```python
from build123d import *

# Parameters (mm, degrees)
BLOCK_BODY_2IN_DEPTH                      = 50.8
SIDE_THROUGH_HOLE_0_234_D                 = 5.9436
SIDE_HOLE_EDGE_CHAMFER_SIZE               = 0.635
DOWEL_HOLE_0_126_D                        = 3.2004
DOWEL_HOLE_0_126_DEPTH                    = 6.0198
DOWEL_HOLE_0_126_TIP                      = 1.6002
COUNTERSUNK_SCREW_HOLE_NO0_D              = 6.7564
COUNTERSUNK_SCREW_HOLE_NO0_CSINK_D        = 13.208
COUNTERSUNK_SCREW_HOLE_NO0_CSINK_ANGLE    = 82
COUNTERBORED_BOLT_HOLE_0_25IN_D           = 6.7564
COUNTERBORED_BOLT_HOLE_0_25IN_CBORE_D     = 11.176
COUNTERBORED_BOLT_HOLE_0_25IN_CBORE_DEPTH = 6.35


with BuildPart() as part:
    # Block Profile Sketch → Block Body 2in (new body)
    with BuildSketch(Plane.XY):
        Polygon((0, 12.7), (19.05, 12.7), (19.05, -31.75), (0, -31.75), (0, 0), (-15.875, 0), (-15.875, 12.7), align=None)
    extrude(amount=BLOCK_BODY_2IN_DEPTH)

    # Side Through Hole Ø0.234 (through all)
    with Locations(Plane(origin=(0, -15.875, 25.4), x_dir=(0, -1, 0), z_dir=(-1, 0, 0))):
        with Locations((0, 0)):
            Hole(SIDE_THROUGH_HOLE_0_234_D / 2)

    # Side Hole Edge Chamfer
    side_hole_edge_chamfer_edges = [part.edges().sort_by_distance(p)[0] for p in [
        (0, -18.8468, 25.4),
        (19.05, -18.8468, 25.4),
    ]]
    chamfer(side_hole_edge_chamfer_edges, length=SIDE_HOLE_EDGE_CHAMFER_SIZE)

    # Dowel Hole Ø0.126
    with Locations(Plane(origin=(-7.9375, 0, 25.4), x_dir=(-1, 0, 0), z_dir=(0, -1, 0))):
        with Locations((0, 0)):
            Hole(DOWEL_HOLE_0_126_D / 2, depth=DOWEL_HOLE_0_126_DEPTH)
            with Locations((0, 0, -(DOWEL_HOLE_0_126_DEPTH + DOWEL_HOLE_0_126_TIP / 2))):  # 90° drill point
                Cone(0, DOWEL_HOLE_0_126_D / 2, DOWEL_HOLE_0_126_TIP, mode=Mode.SUBTRACT)

    # Countersunk Screw Hole No0 (through all)
    with Locations(Plane(origin=(-7.9375, 12.7, 12.7), x_dir=(0, 0, 1), z_dir=(0, 1, 0))):
        with Locations((0, 0)):
            CounterSinkHole(COUNTERSUNK_SCREW_HOLE_NO0_D / 2, COUNTERSUNK_SCREW_HOLE_NO0_CSINK_D / 2, counter_sink_angle=COUNTERSUNK_SCREW_HOLE_NO0_CSINK_ANGLE)

    # Counterbored Bolt Hole 0.25in (through all)
    with Locations(Plane(origin=(-7.9375, 12.7, 38.1), x_dir=(0, 0, 1), z_dir=(0, 1, 0))):
        with Locations((0, 0)):
            CounterBoreHole(COUNTERBORED_BOLT_HOLE_0_25IN_D / 2, COUNTERBORED_BOLT_HOLE_0_25IN_CBORE_D / 2, COUNTERBORED_BOLT_HOLE_0_25IN_CBORE_DEPTH)


solid = part.part
```
Model file for the job. Use its own axes, mm. A direction names the side the tool comes from. Coordinates: 2 decimals unless noted, no trailing zeros. Order: outer loops, then holes, each group sorted by start corner. A loop starts at its lowest first (then second) coordinate and runs counter-clockwise, first axis right, second up. Notation, with made-up numbers: (59.5, 62) -> (69.5, 62) arc R21 cw to (69.5, 74) -> close; hole circle Ø5 at (52, 57.25). An arc over 180 degrees is marked (long way). Answer as a JSON object with one key per item and string values. Group by question number.
1) Cut at D-D, the plane z = 31.5. Write the cut outline in (x, y) (3 decimals).
2) Cut at B-B, the plane y = 2.5. Count the separate pieces of the cut face and the enclosed holes in it, then the cut area to 3 significant figures.
3) Flat gauge pins, fed straight in: pin 1 (8 mm diameter, centred on x = -7.94, z = 38.1, fed in from -Y); pin 2 (17.5 mm diameter, centred on x = -4.5, z = 30, fed in from -Y); pin 3 (2 mm diameter, centred on y = -15.5, z = 5.5, fed in from -X); pin 4 (8 mm diameter, centred on x = -7.94, z = 12.7, fed in from +Y). Where does each tip first touch, or does it go through?
4) Drill centre lines: L1, parallel to X at y = 3.5, z = 25.4 (3 decimals); L2, parallel to X at y = 6, z = 13 (3 decimals); L3, parallel to X at y = -14.5, z = 46.5. Where is each one in solid material? Low to high.
5) Which spindle directions (+Z, -Z, +X, -X, +Y, -Y) get a long thin tool onto all of the face, cutting with end or side? Do faces 1 (the face through (-7.789, 3.131, 41.475)), 2 (the face through (-6, 0, 25)), 3 (the face through (-8.146, 3.052, 23.813)), 4 (the face through (-10, 6.35, 41)), 5 (the face through (-15.875, 6, 25)). Say none if no direction does.
6) Pull direction X, two halves, no side cores. Call faces 6 (the face through (10, -31.75, 25)), 7 (the face through (19.05, -9, 25)), 8 (the face through (-7.78, 9.17, 16.23)): +X half, -X half, draft (parallel to the pull), parting line (faces both ways), or undercut.
Check values:
{
 "1": {"outline": "(-15.875, 0) -> (0, 0) -> (0, -31.75) -> (19.05, -31.75) -> (19.05, 12.7) -> (-15.875, 12.7) -> close"},
 "2": {"separate pieces": "1", "enclosed holes": "3", "area": "1,690 mm²"},
 "3": {"pin 1": "stops at y = 0", "pin 2": "stops at y = -31.75", "pin 3": "stops at x = 0", "pin 4": "stops at y = 9.71"},
 "4": {"L1": "x = -15.875 to -9.538, -6.337 to 19.05", "L2": "x = -15.875 to -11.302, -4.573 to 19.05", "L3": "x = 0 to 19.05"},
 "5": {"face 1": "+Y, -Y", "face 2": "+Z, -Z, -X, -Y", "face 3": "-Y", "face 4": "+Y", "face 5": "+Z, -Z, -X, +Y, -Y"},
 "6": {"face 6": "draft", "face 7": "+X half", "face 8": "undercut"}
}
